Drawing for the job (mm, zero at the part's lowest x, y, z). A direction names the side the tool comes from. Coordinates: 2 decimals unless noted, no trailing zeros. Loops run counter-clockwise (first coordinate to the right, second up) from the corner with the lowest first, then second, coordinate; pieces in that order, holes last.
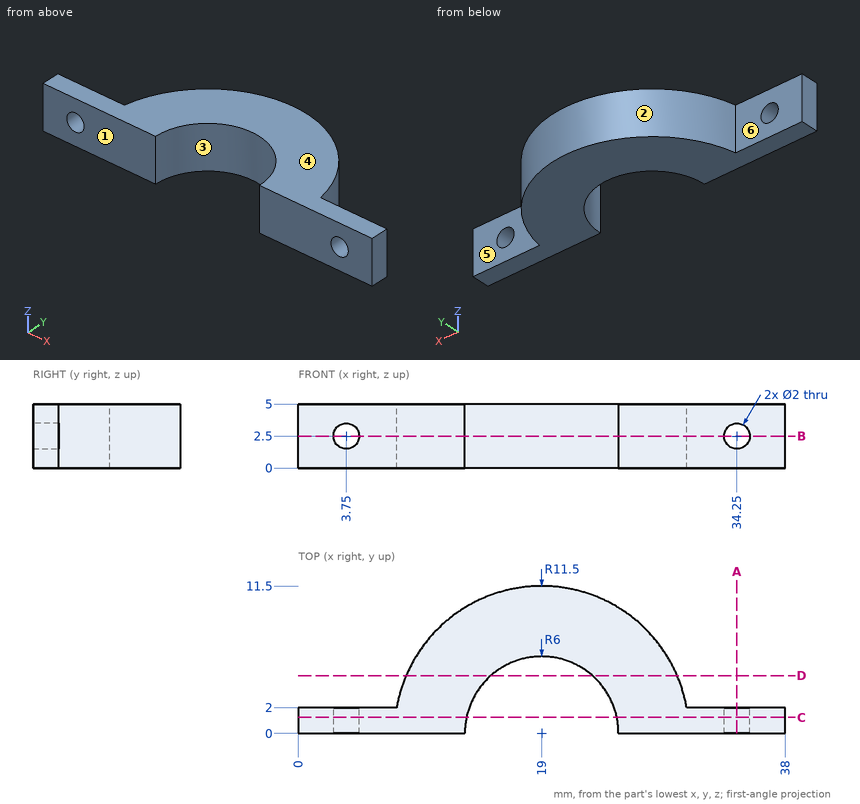
Q1. Saw through at B-B (z = 2.5). List the corners of the cut face in (x, y).
Q2. Tool access for the marked faces 4, 5 and 6: list every direction of +Z, -Z, +X, -X, +Y, -Y with a clear straight run to the whole face (end or side of a thin tool).
Q3. Saw through at C-C (y = 1.25). List the corners of the cut face in (x, z), plus the area to 3 significant figures.
Q4. Mould opens along X. For the marked faces 1, 2 and 3 say: released by +X, released by -X, zero draft, split by the parting line, or undercut.
Q5. Probe line 1 (X direction, y = 1.4, z = 2.5); line 2 (X direction, y = 0.5, z = 2.5); line 3 (Y direction, x = 6, z = 2.65). List the from-to ranges inside material, lowest first.
Q6. Saw through at A-A (x = 34.25). List the corners of the cut face in (y, z), plus the area to 3 significant figures.
Q7. Saw through at D-D (y = 4.5). List the corners of the cut face in (x, z).
Q8. Drop flat-ended pins along their axis: P1, Ø1.5, axis at y = 4.5, z = 1, coming from the -X side; P2, Ø2.5, axis at x = 3.75, z = 2.5, coming from the +Y side; P3, Ø1.5, axis at y = 7.5, z = 4, coming from the -X side. Give the stop position or say it passes through.
Checked values:
1. outline: (0, 0) - (2.75, 0) - (2.75, 2) - (0, 2) - close; (4.75, 0) - (13, 0) arc R6 cw to (25, 0) - (33.25, 0) - (33.25, 2) - (30.32, 2) arc R11.5 ccw to (7.68, 2) - (4.75, 2) - close; (35.25, 0) - (38, 0) - (38, 2) - (35.25, 2) - close
2. face 4: +Z, +X, -X, +Y, -Y
2. face 5: +Z, -Z, +X, +Y
2. face 6: +Z, -Z, -X, +Y
3. outline: (0, 0) - (13.13, 0) - (13.13, 5) - (0, 5) - close; (24.87, 0) - (38, 0) - (38, 5) - (24.87, 5) - close; hole circle Ø2 at (3.75, 2.5); hole circle Ø2 at (34.25, 2.5)
3. area: 125 mm2
4. face 1: zero draft
4. face 2: split by the parting line
4. face 3: undercut
5. line 1: x = 0 to 2.75, 4.75 to 13.17, 24.83 to 33.25, 35.25 to 38
5. line 2: x = 0 to 2.75, 4.75 to 13.02, 24.98 to 33.25, 35.25 to 38
5. line 3: y = 0 to 2
6. outline: (0, 0) - (2, 0) - (2, 1.5) - (0, 1.5) - close; (0, 3.5) - (2, 3.5) - (2, 5) - (0, 5) - close
6. area: 6.00 mm2
7. outline: (8.42, 0) - (15.03, 0) - (15.03, 5) - (8.42, 5) - close; (22.97, 0) - (29.58, 0) - (29.58, 5) - (22.97, 5) - close
8. P1: stops at x = 8.13
8. P2: stops at y = 2
8. P3: stops at x = 9.69
